from build123d import *

# Parameters (mm, degrees)
SKETCH1_R           = 52
SKETCH1_R_2         = 20
BOSS_EXTRUDE1_DEPTH = 30


with BuildPart() as part:
    # Sketch1 → Boss-Extrude1 (new body)
    with BuildSketch(Plane.XY):
        Circle(SKETCH1_R)
        Circle(SKETCH1_R_2, mode=Mode.SUBTRACT)
    extrude(amount=BOSS_EXTRUDE1_DEPTH)

    # Sketch2 → Cut-Revolve1 (revolve, cut)
    with BuildSketch(Plane(origin=(0, 0, 0), x_dir=(0, 0, -1), z_dir=(1, 0, 0)), mode=Mode.PRIVATE) as cut_revolve1_sk:
        Polygon((-25.316178594, 46), (-19.683821406, 46), (-17.5, 52), (-27.5, 52), align=None)
        Polygon((-12.5, 52), (-10.316178594, 46), (-4.683821406, 46), (-2.5, 52), align=None)
    revolve(cut_revolve1_sk.sketch.rotate(Axis((0, 0, 0), (0, 0, 1)), 90), axis=Axis((0, 0, 0), (0, 0, 1)), mode=Mode.SUBTRACT)


solid = part.part
Build history of the part. All positions in model axes, mm. A direction names the side the tool comes from. Round coordinates to 2 decimals unless told otherwise and drop trailing zeros. Write each loop counter-clockwise with the first axis right and the second up, starting at its lowest first coordinate (ties: lowest second). Pieces come first, ordered by that corner, then holes. Notation, with made-up numbers: (39.5, 51.5) - (97.5, 51.5) arc R14 cw to (97.5, 56.5) - close; hole circle Ø9 at (19, 86). An arc over 180 degrees is marked (long way). One line per question, with ' | ' between items.
1. Band-saw the part on A-A, the plane x = 0. Write the cut outline in (y, z).
Results are:
outline: (-52, 0) - (-20, 0) - (-20, 30) - (-52, 30) - (-52, 27.5) - (-46, 25.32) - (-46, 19.68) - (-52, 17.5) - (-52, 12.5) - (-46, 10.32) - (-46, 4.68) - (-52, 2.5) - close; (20, 0) - (52, 0) - (52, 2.5) - (46, 4.68) - (46, 10.32) - (52, 12.5) - (52, 17.5) - (46, 19.68) - (46, 25.32) - (52, 27.5) - (52, 30) - (20, 30) - close
2. Drill centre lines: line 1 along Y through (x, z) = (0, 15); line 2 along Z through (x, y) = (46, -6.5); line 3 along Y through (x, z) = (-9.5, 13.5). Where is each one in solid material? Low to high. Write a range as from..to.
Results are:
line 1: -52..-20, 20..52 | line 2: 0..4.52, 10.48..19.52, 25.48..30 | line 3: -51.12..-17.6, 17.6..51.12
3. Tool access for faces 5 (the face through (-41.265, -31.641, 14.965)), 6 (the face through (5.99, -45.61, 22.46)): list every direction of +Z, -Z, +X, -X, +Y, -Y with a clear straight run to the whole face (end or side of a thin tool).
Results are:
face 5: +Z, -Z | face 6: none
4. Drop flat-ended pins along their axis: pin 1 Ø5 at (y, z) = (-7, 16.5) entering from +X; pin 2 Ø1 at (x, z) = (34, 23) entering from -Y; pin 3 Ø2 at (y, z) = (-17.5, 9) entering from -X. Give the stop position or say it passes through.
Results are:
pin 1: x = 51.8 | pin 2: y = -31.52 | pin 3: x = -42.94
5. Mould opens along Z. For faces 1 (the face through (22, 1, 0)), 2 (the face through (-41.265, -31.641, 1.232)), 3 (the face through (22, 1, 30)), 4 (the face through (-44.23, -13.93, 4.55)) say: released by +Z, released by -Z, zero draft, split by the parting line, or undercut.
Results are:
face 1: released by -Z | face 2: zero draft | face 3: released by +Z | face 4: undercut
